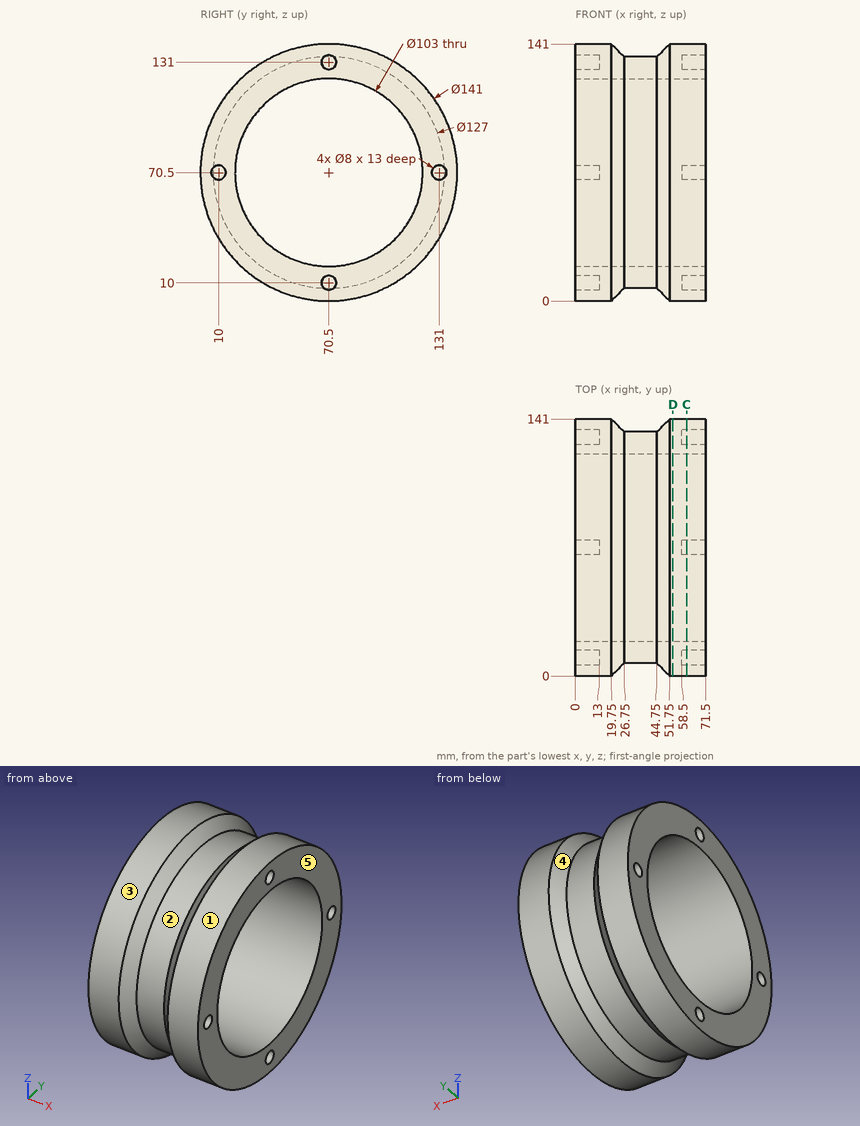
Geometry: see drawing. Coordinates: mm, zero at the bounding-box minimum. A direction names the side the tool comes from. Coordinates: 2 decimals unless noted, no trailing zeros. Order: outer loops, then holes, each group sorted by start corner. A loop starts at its lowest first (then second) coordinate and runs counter-clockwise, first axis right, second up. Notation, with made-up numbers: (80.25, -30) - (130.25, -30) arc R32 cw to (130.25, -1) - close; hole circle Ø3 at (61, -2). An arc over 180 degrees is marked (long way). Write each question's results on one line, items separated by ' | '.
(1) Section query D-D, the plane x = 53.5. Return the cut outline in (y, z), plus the area to 3 significant figures.
Values found:
outline: circle Ø141 at (70.5, 70.5); hole circle Ø103 at (70.5, 70.5) | area: 7,280 mm²
(2) First-contact query: pin 1 Ø6.5 at (y, z) = (131, 70.5) entering from -X; pin 2 Ø1.5 at (x, z) = (43.5, 77.5) entering from +Y; pin 3 Ø1.5 at (y, z) = (20, 18.5) entering from -X; pin 4 Ø7 at (y, z) = (10, 70.5) entering from +X. Flat tips, straight axial feed; report the tip coordinate or a pass-through.
Values found:
pin 1: stops at x = 13 | pin 2: stops at y = 133.69 | pin 3: passes through | pin 4: stops at x = 58.5
(3) Mould query, pull axis X, two halves, no side actions, for the marked faces 3, 4 and 5. Classes: +X half, -X half, draft (parallel to the pull), parting line (faces both ways), or undercut.
Values found:
face 3: draft | face 4: undercut | face 5: +X half
(4) Line query: line 1 (Y direction, x = 5.5, z = 70.5); line 2 (Y direction, x = 34, z = 71). Output: solid intervals per line, ascending. Write a range as [from, to].
Values found:
line 1: y = [0, 6], [14, 19], [122, 127], [135, 141] | line 2: y = [7, 19], [122, 134]
(5) Set-up query: the marked faces 1 and 2. Return all of +Z, -Z, +X, -X, +Y, -Y with unobstructed straight access to the full face (end or side cutting, diameter ignored); none if empty.
Values found:
face 1: +X, -X | face 2: none
(6) Section query C-C, the plane x = 61. Return the cut outline in (y, z), plus the area to 3 significant figures.
Values found:
outline: circle Ø141 at (70.5, 70.5); hole circle Ø8 at (10, 70.5); hole circle Ø103 at (70.5, 70.5); hole circle Ø8 at (70.5, 10); hole circle Ø8 at (70.5, 131); hole circle Ø8 at (131, 70.5) | area: 7,080 mm²
